```python
from build123d import *

# Parameters (mm, degrees)
BRACKET_BODY_DEPTH        = 2.5
FACE_RECESS_SKETCH_R      = 1.4
FACE_RECESS_2_8X1_DEPTH   = 1
MOUNTING_HOLES_SKETCH_R   = 0.5
FOOT_MOUNTING_HOLES_DEPTH = 12.456439237
CORNER_FILLETS_R1_R       = 1
RECESS_EDGE_FILLET_R0_2_R = 0.2


with BuildPart() as part:
    # Bracket Profile Sketch → Bracket Body (new, symmetric)
    with BuildSketch(Plane.XY):
        with BuildLine():
            Line((0, 1), (0, 6))
            Line((0, 6), (1, 6))
            Line((1, 6), (5, 1))
            Line((5, 1), (10, 1))
            Line((10, 1), (10, 0))
            Line((10, 0), (1, 0))
            ThreePointArc((1, 0), (0.292893219, 0.292893219), (0, 1))
        make_face()
    extrude(amount=BRACKET_BODY_DEPTH, both=True)

    # Face Recess Sketch → Face Recess Ø2.8x1 (cut)
    with BuildSketch(Plane(origin=(3.536585366, 2.829268293, 0), x_dir=(0, 0, -1), z_dir=(0.7808688094430304, 0.6246950475544242, 0))):
        with Locations(Location((0, 0, 0), (0, 0, 90))):
            Circle(FACE_RECESS_SKETCH_R)
    extrude(amount=-FACE_RECESS_2_8X1_DEPTH, mode=Mode.SUBTRACT)

    # Mounting Holes Sketch → Foot Mounting Holes (cut, through all)
    with BuildSketch(Plane(origin=(0, 1, 0), x_dir=(1, 0, 0), z_dir=(0, 1, 0))):
        with Locations(Location((9, -1.5, 0), (0, 0, 270))):
            Circle(MOUNTING_HOLES_SKETCH_R)
        with Locations(Location((9, 1.5, 0), (0, 0, 270))):
            Circle(MOUNTING_HOLES_SKETCH_R)
    extrude(amount=-FOOT_MOUNTING_HOLES_DEPTH, mode=Mode.SUBTRACT)

    # Corner Fillets R1
    corner_fillets_r1_edges = [part.edges().sort_by_distance(p)[0] for p in [
        (10, 0.5, 2.5),
        (10, 0.5, -2.5),
    ]]
    fillet(corner_fillets_r1_edges, radius=CORNER_FILLETS_R1_R)

    # Recess Edge Fillet R0.2
    recess_edge_fillet_r0_2_edges = [part.edges().sort_by_distance(p)[0] for p in [
        (3.630289623, 1.111356912, 0),
    ]]
    fillet(recess_edge_fillet_r0_2_edges, radius=RECESS_EDGE_FILLET_R0_2_R)


solid = part.part
```
Work out the finished part from the listing and answer in its coordinate system (mm). A direction names the side the tool comes from. Coordinates: 2 decimals unless noted, no trailing zeros. Loops run counter-clockwise (first coordinate to the right, second up) from the corner with the lowest first, then second, coordinate; pieces in that order, holes last.
1) Section B-B (y = 5.25) is taken. Give the vertices of the cut face in (x, z).
Results:
outline: (0, -2.5) - (1.6, -2.5) - (1.6, 2.5) - (0, 2.5) - close
2) For a pull along Z with two mould halves and no side action, classify faces 1 (the cylindrical face through (8.512, 0.507, -1.608)), 2 (the flat face through (3, 2, 2.5)), 3 (the cylindrical face through (9.699, 0.493, -2.215)), 4 (the flat face through (2.53, 4.09, 0.04)) as +Z half, -Z half, draft (parallel to the pull), parting line (faces both ways), or undercut.
Results:
face 1: undercut
face 2: +Z half
face 3: -Z half
face 4: draft
3) Section A-A (x = 6.25) is taken. Give the vertices of the cut face in (y, z).
Results:
outline: (0, -2.5) - (1, -2.5) - (1, 2.5) - (0, 2.5) - close
4) For faces 5 (the flat face through (2.766, 2.191, 0.017)), 6 (the flat face through (7, 1, 0)), 7 (the cylindrical face through (9.699, 0.493, 2.215)), determine the directions among +Z, -Z, +X, -X, +Y, -Y from which every point of the face is accessible in a straight line to the end or side of a thin tool.
Results:
face 5: none
face 6: +Z, -Z, +X, +Y
face 7: +Z, +X, +Y, -Y
5) A flat-ended cylindrical pin translates along its axis: pin 1 (3 mm diameter, centred on y = 3.5, z = -0.5, fed in from +X). Find the tip coordinate at first contact, or state that the pin passes through.
Results:
pin 1: stops at x = 4.12
6) Consider probe 1 along Y at (x, z) = (8.5, 1.7); probe 2 along X at (y, z) = (0.7, -1.5); probe 3 along Z at (x, y) = (2.75, 2.45). Determine where each line is inside the solid, lowest interval first.
Results:
probe 1: y = 0 to 1
probe 2: x = 0.05 to 8.5, 9.5 to 10
probe 3: z = -2.5 to -1.38, 1.38 to 2.5
